```python
from build123d import *

# Parameters (mm, degrees)
SKETCH1_W           = 10
SKETCH1_H           = 10
SKETCH1_W_2         = 9
SKETCH1_H_2         = 9
BOSS_EXTRUDE1_DEPTH = 355
SKETCH2_R           = 4
BOSS_EXTRUDE2_DEPTH = 8
SKETCH3_R           = 3
BOSS_EXTRUDE3_DEPTH = 2
SKETCH4_R           = 4
BOSS_EXTRUDE4_DEPTH = 3
SKETCH5_R           = 3
CUT_EXTRUDE1_DEPTH  = 21
SKETCH6_R           = 3
CUT_EXTRUDE2_DEPTH  = 18


with BuildPart() as part:
    # Sketch1 → Boss-Extrude1 (new body)
    with BuildSketch(Plane(origin=(0, 0, 0), x_dir=(1, 0, 0), z_dir=(0, 1, 0))):
        Rectangle(SKETCH1_W, SKETCH1_H)
        Rectangle(SKETCH1_W_2, SKETCH1_H_2, mode=Mode.SUBTRACT)
    extrude(amount=BOSS_EXTRUDE1_DEPTH)

    # Sketch2 → Boss-Extrude2 (add)
    with BuildSketch(Plane(origin=(5, 0, 0), x_dir=(0, 0, -1), z_dir=(1, 0, 0))):
        with Locations(Location((0, 193, 0), (0, 0, 180))):
            Circle(SKETCH2_R)
    extrude(amount=BOSS_EXTRUDE2_DEPTH)

    # Sketch3 → Boss-Extrude3 (add)
    with BuildSketch(Plane(origin=(13, 0, 0), x_dir=(0, 0, -1), z_dir=(1, 0, 0))):
        with Locations((0, 193)):
            Circle(SKETCH3_R)
    extrude(amount=BOSS_EXTRUDE3_DEPTH)

    # Sketch4 → Boss-Extrude4 (add)
    with BuildSketch(Plane(origin=(15, 0, 0), x_dir=(0, 0, -1), z_dir=(1, 0, 0))):
        with Locations(Location((0, 193, 0), (0, 0, 180))):
            Circle(SKETCH4_R)
    extrude(amount=BOSS_EXTRUDE4_DEPTH)

    # Mirror1: part across plane


with BuildPart() as part_1:
    add(part.part)
    add(part.part.mirror(Plane(origin=(0, 0, 0), x_dir=(0, 0, 1), z_dir=(1, 0, 0))))

    # Sketch5 → Cut-Extrude1 (cut)
    with BuildSketch(Plane(origin=(5, 0, 0), x_dir=(0, 0, -1), z_dir=(1, 0, 0))):
        with Locations((0, 5)):
            Circle(SKETCH5_R)
    extrude(amount=-CUT_EXTRUDE1_DEPTH, mode=Mode.SUBTRACT)

    # Sketch6 → Cut-Extrude2 (cut)
    with BuildSketch(Plane.ZY.offset(5)):
        with Locations((0, 350)):
            Circle(SKETCH6_R)
    extrude(amount=-CUT_EXTRUDE2_DEPTH, mode=Mode.SUBTRACT)


solid = part_1.part
```
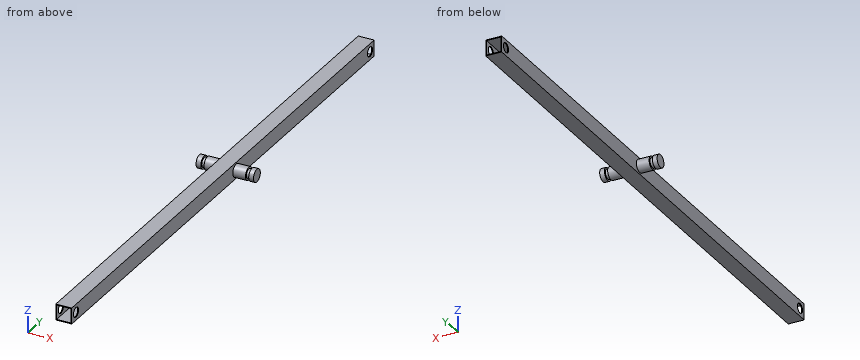
Geometry check sheet. Reference: the model listing, model coordinates, mm. Round coordinates to 2 decimals unless told otherwise and drop trailing zeros. Order: outer loops, then holes, each group sorted by start corner. A loop starts at its lowest first (then second) coordinate and runs counter-clockwise, first axis right, second up. Notation, with made-up numbers: (86, 37.25) -> (92, 37.25) arc R17 ccw to (92, 68.25) -> close; hole circle Ø11 at (53, 41). An arc over 180 degrees is marked (long way). Return JSON: item names as keys, results as strings. Group by question number.
Q1. Section check A-A, the plane x = -0.5. Record the boundary of the cut face in (y, z).
Q2. Section check D-D, the plane z = 0. Count the separate pieces of the cut face and the enclosed holes in it, plus the area to 3 significant figures.
Q3. Material ranges on probe 1 along Y at (x, z) = (4.8, 0); probe 2 along Z at (x, y) = (-3, 312), recorded low to high. Write a range as from..to.
Q4. Section check B-B, the plane y = 350. Record the boundary of the cut face in (x, z), plus the area to 3 significant figures.
Q5. Gauge pin test, flat ends, axial feed: pin 1 (1 mm diameter, centred on x = 8.5, z = 3, fed in from +Y); pin 2 (3 mm diameter, centred on y = 129.5, z = 1, fed in from +X); pin 3 (5 mm diameter, centred on y = 203, z = 0.5, fed in from -X); pin 4 (5 mm diameter, centred on y = 5, z = 0, fed in from -X). Record the tip position at first contact, or that the pin passes through.
Numbers:
{
 "1": {"outline": "(0, -5) -> (355, -5) -> (355, -4.5) -> (0, -4.5) -> close; (0, 4.5) -> (355, 4.5) -> (355, 5) -> (0, 5) -> close"},
 "2": {"separate pieces": "6", "enclosed holes": "0", "area": "543 mm^2"},
 "3": {"probe 1": "0..2, 8..347, 353..355", "probe 2": "-5..-4.5, 4.5..5"},
 "4": {"outline": "(-5, -5) -> (5, -5) -> (5, -3) -> (4.5, -3) -> (4.5, -4.5) -> (-4.5, -4.5) -> (-4.5, -3) -> (-5, -3) -> close; (-5, 3) -> (-4.5, 3) -> (-4.5, 4.5) -> (4.5, 4.5) -> (4.5, 3) -> (5, 3) -> (5, 5) -> (-5, 5) -> close", "area": "13.0 mm^2"},
 "5": {"pin 1": "y = 196.12", "pin 2": "x = 5", "pin 3": "x = -5", "pin 4": "through"}
}
